The model under review builds one solid part; all positions refer to its coordinate system, in mm. A direction names the side the tool comes from. Coordinates: 2 decimals unless noted, no trailing zeros. Write each loop counter-clockwise with the first axis right and the second up, starting at its lowest first coordinate (ties: lowest second). Pieces come first, ordered by that corner, then holes. Notation, with made-up numbers: (32.25, -7) - (53.25, -7) arc R23 ccw to (53.25, 18) - close; hole circle Ø10 at (-11.5, 43.25). An arc over 180 degrees is marked (long way). Answer as CSV lines item,"result". Start each with the question number.
```python
from build123d import *

# Parameters (mm, degrees)
SKETCH1_W           = 25
SKETCH1_H           = 12
BOSS_EXTRUDE1_DEPTH = 25
CUT_EXTRUDE1_DEPTH  = 30
CHAMFER1_SIZE       = 2
SKETCH5_W           = 21
SKETCH5_H           = 35
BOSS_EXTRUDE2_DEPTH = 6
SKETCH6_W           = 2.6
SKETCH6_H           = 5
CUT_EXTRUDE2_DEPTH  = 10
SKETCH11_W          = 14.4
SKETCH11_H          = 0.3
CUT_EXTRUDE5_DEPTH  = 48
CUT_EXTRUDE6_DEPTH  = 48
SKETCH15_W          = 25
SKETCH15_H          = 12
CUT_EXTRUDE8_DEPTH  = 0.5
SKETCH17_R          = 2
CUT_EXTRUDE10_DEPTH = 5
SKETCH18_R          = 1
CUT_EXTRUDE11_DEPTH = 4
CUT_EXTRUDE12_DEPTH = 17
CUT_EXTRUDE13_DEPTH = 9


with BuildPart() as part:
    # Sketch1 → Boss-Extrude1 (new body)
    with BuildSketch(Plane.XY):
        with Locations((12.5, -6)):
            Rectangle(SKETCH1_W, SKETCH1_H)
    extrude(amount=BOSS_EXTRUDE1_DEPTH)

    # Sketch2 → Cut-Extrude1 (cut)
    with BuildSketch(Plane.XY.offset(25)):
        Polygon((25, 0), (25, -7.967433715), (20.4, 0), align=None)
    extrude(amount=-CUT_EXTRUDE1_DEPTH, mode=Mode.SUBTRACT)

    # Chamfer1
    chamfer1_edges = [part.edges().sort_by_distance(p)[0] for p in [
        (0, 0, 12.5),
        (25, -12, 12.5),
        (0, -12, 12.5),
    ]]
    chamfer(chamfer1_edges, length=CHAMFER1_SIZE)

    # Sketch5 → Boss-Extrude2 (add)
    with BuildSketch(Plane.XZ.offset(12)):
        with Locations((12.5, 12.5)):
            Rectangle(SKETCH5_W, SKETCH5_H)
    extrude(amount=-BOSS_EXTRUDE2_DEPTH)

    # Sketch6 → Cut-Extrude2 (cut)
    with BuildSketch(Plane(origin=(0, -6, 0), x_dir=(1, 0, 0), z_dir=(0, 1, 0))):
        with Locations((21.7, -27.5)):
            Rectangle(SKETCH6_W, SKETCH6_H)
        with Locations((21.7, 2.5)):
            Rectangle(SKETCH6_W, SKETCH6_H)
    extrude(amount=-CUT_EXTRUDE2_DEPTH, mode=Mode.SUBTRACT)

    # Sketch11 → Cut-Extrude5 (cut)
    with BuildSketch(Plane.XY.offset(30)):
        with Locations((11.2, -11.85)):
            Rectangle(SKETCH11_W, SKETCH11_H)
    extrude(amount=-CUT_EXTRUDE5_DEPTH, mode=Mode.SUBTRACT)

    # Sketch12 → Cut-Extrude6 (cut)
    with BuildSketch(Plane.XY.offset(30)):
        Polygon((25, -7.967433715), (20.4, -12), (25.592855108, -12), align=None)
    extrude(amount=-CUT_EXTRUDE6_DEPTH, mode=Mode.SUBTRACT)

    # Sketch15 → Cut-Extrude8 (cut)
    with BuildSketch(Plane.ZY):
        with Locations((12.5, -6)):
            Rectangle(SKETCH15_W, SKETCH15_H)
    extrude(amount=-CUT_EXTRUDE8_DEPTH, mode=Mode.SUBTRACT)

    # Sketch17 → Cut-Extrude10 (cut)
    with BuildSketch(Plane(origin=(0, 0, 0), x_dir=(1, 0, 0), z_dir=(0, 1, 0))):
        with Locations(Location((11.2, -6.7, 0), (0, 0, 270))):
            Circle(SKETCH17_R)
        with Locations(Location((11.2, -18.3, 0), (0, 0, 270))):
            Circle(SKETCH17_R)
    extrude(amount=-CUT_EXTRUDE10_DEPTH, mode=Mode.SUBTRACT)

    # Sketch18 → Cut-Extrude11 (cut)
    with BuildSketch(Plane(origin=(0, 0, 0), x_dir=(1, 0, 0), z_dir=(0, 1, 0))):
        with Locations(Location((4.7, -12.5, 0), (0, 0, 270))):
            Circle(SKETCH18_R)
        with Locations(Location((17.7, -12.5, 0), (0, 0, 270))):
            Circle(SKETCH18_R)
    extrude(amount=-CUT_EXTRUDE11_DEPTH, mode=Mode.SUBTRACT)

    # Sketch19 → Cut-Extrude12 (cut)
    with BuildSketch(Plane(origin=(0, 0, 0), x_dir=(1, 0, 0), z_dir=(0, 1, 0))):
        with BuildLine():
            Line((12.9, -25), (12.9, -28))
            ThreePointArc((12.9, -28), (11.2, -29.7), (9.5, -28))
            Line((9.5, -28), (9.5, -25))
            ThreePointArc((9.5, -25), (11.2, -23.3), (12.9, -25))
        make_face()
        with BuildLine():
            Line((12.9, 0), (12.9, 3))
            ThreePointArc((12.9, 3), (11.2, 4.7), (9.5, 3))
            Line((9.5, 3), (9.5, 0))
            ThreePointArc((9.5, 0), (11.2, -1.7), (12.9, 0))
        make_face()
    extrude(amount=-CUT_EXTRUDE12_DEPTH, mode=Mode.SUBTRACT)

    # Sketch20 → Cut-Extrude13 (cut)
    with BuildSketch(Plane(origin=(0, 0, 0), x_dir=(1, 0, 0), z_dir=(0, 1, 0))):
        with BuildLine():
            Line((14.4, -25), (14.4, -28))
            ThreePointArc((14.4, -28), (11.2, -31.2), (8, -28))
            Line((8, -28), (8, -25))
            ThreePointArc((8, -25), (11.2, -21.8), (14.4, -25))
        make_face()
        with BuildLine():
            Line((14.4, 0), (14.4, 3))
            ThreePointArc((14.4, 3), (11.2, 6.2), (8, 3))
            Line((8, 3), (8, 0))
            ThreePointArc((8, 0), (11.2, -3.2), (14.4, 0))
        make_face()
    extrude(amount=-CUT_EXTRUDE13_DEPTH, mode=Mode.SUBTRACT)


solid = part.part
```
(1) Add section A-A on z = 14.5. Give the boundary of the cut face in (x, y).
(2) Add section D-D on x = 23. Give the boundary of the cut face in (y, z), then the cut area to 3 significant figures.
(3) Wall thickness on line 1 (X direction, y = -1.8, z = 12.5); line 2 (Z direction, x = 12, y = -3.75); line 3 (X direction, y = -8, z = 27): over which ranges is each line inside the solid? List them lowest first.
(4) The part is to be moulded in two halves that separate along X. For faces 1 (the flat face through (18, -4, 12)), 2 (the flat face through (5, -6, -2)), 3 (the flat face through (0.5, -6, 12)), say which applies: released by +X, released by -X, zero draft, split by the parting line, or undercut.
(5) For faces 4 (the cylindrical face through (11.2, -10.3, 29.7)), 5 (the cylindrical face through (14.224, -7.479, 29.046)), 6 (the flat face through (11, -10, -5)), list the 3-axis set-ups (+Z, -Z, +X, -X, +Y, -Y) from which the entire face can be reached by the end or side of a thin tool; tool diameter is ignored.
(6) Add section B-B on y = -1. Give the boundary of the cut face in (x, z), then the cut area to 3 significant figures.
(7) For pin 1 (2 mm diameter, centred on x = 21.5, y = -2.5, fed in from -Z); pin 2 (2.5 mm diameter, centred on x = 18, z = -2.5, fed in from +Y); pin 3 (1.5 mm diameter, centred on y = -10, z = -2, fed in from -X), all flat-tipped, find the tip position at first contact; note any pin that passes through.
(8) Add section C-C on y = -6.5. Give the boundary of the cut face in (x, z), then the cut area to 3 significant figures.
Reported:
1,outline,"(0.5, -10.5) - (2, -12) - (4, -12) - (4, -11.7) - (18.4, -11.7) - (18.4, -12) - (20.4, -12) - (25, -7.97) - (20.4, 0) - (2, 0) - (0.5, -1.5) - close"
2,outline,"(-9.72, 0) - (-4.5, 0) - (-4.5, 25) - (-9.72, 25) - close"
2,area,"130 mm²"
3,line 1,"0.5 to 3.7, 5.7 to 16.7, 18.7 to 21.44"
3,line 2,"3.1 to 4.87, 8.53 to 16.47, 20.13 to 21.9"
3,line 3,"2 to 8, 14.4 to 20.4"
4,face 1,"undercut"
4,face 2,"zero draft"
4,face 3,"released by -X"
5,face 4,"+Y, -Y"
5,face 5,"+Y"
5,face 6,"-Z, +X, -X, +Y, -Y"
6,outline,"(1, 0) - (8, 0) arc R3.2 cw to (14.4, 0) - (20.98, 0) - (20.98, 25) - (14.4, 25) arc R3.2 cw to (8, 25) - (1, 25) - close; hole circle Ø2 at (4.7, 12.5); hole circle Ø4 at (11.2, 6.7); hole circle Ø4 at (11.2, 18.3); hole circle Ø2 at (17.7, 12.5)"
6,area,"436 mm²"
7,pin 1,"z = 0"
7,pin 2,"y = -6"
7,pin 3,"x = 2"
8,outline,"(0.5, 0) - (2, 0) - (2, -5) - (8.7, -5) arc R3.2 cw to (8, -3) - (8, 0) arc R3.2 cw to (14.4, 0) - (14.4, -3) arc R3.2 cw to (13.7, -5) - (20.4, -5) - (20.4, 0) - (24.15, 0) - (24.15, 25) - (20.4, 25) - (20.4, 30) - (13.7, 30) arc R3.2 cw to (14.4, 28) - (14.4, 25) arc R3.2 cw to (8, 25) - (8, 28) arc R3.2 cw to (8.7, 30) - (2, 30) - (2, 25) - (0.5, 25) - close"
8,area,"681 mm²"
